For this review, take the finished solid that the model builds, in its own axes (mm). A direction names the side the tool comes from. Give positions to 0.01 mm unless a question says otherwise; leave off trailing zeros. Loops run counter-clockwise (first coordinate to the right, second up) from the corner with the lowest first, then second, coordinate; pieces in that order, holes last. Notation, with made-up numbers: (87, 74) - (106, 74) arc R27 cw to (106, 102) - close; hole circle Ø7 at (1, 60). An arc over 180 degrees is marked (long way). Answer as CSV lines item,"result".
from build123d import *

# Parameters (mm, degrees)
SKETCH1_R           = 12.5
BOSS_EXTRUDE1_DEPTH = 5
SKETCH2_R           = 10
BOSS_EXTRUDE2_DEPTH = 20
CUT_EXTRUDE2_DEPTH  = 3


with BuildPart() as part:
    # Sketch1 → Boss-Extrude1 (new body)
    with BuildSketch(Plane.XY):
        Circle(SKETCH1_R)
    extrude(amount=BOSS_EXTRUDE1_DEPTH)

    # Sketch2 → Boss-Extrude2 (add)
    with BuildSketch(Plane.XY.offset(5)):
        Circle(SKETCH2_R)
    extrude(amount=BOSS_EXTRUDE2_DEPTH)

    # Sketch3 → Cut-Extrude2 (cut)
    with BuildSketch(Plane(origin=(0, 0, 0), x_dir=(-1, 0, 0), z_dir=(0, 0, -1))):
        with BuildLine():
            Line((1.83229916, 12.364977953), (1.83229916, -12.364977953))
            ThreePointArc((1.83229916, -12.364977953), (0, -12.5), (-1.83229916, -12.364977953))
            Line((-1.83229916, -12.364977953), (-1.83229916, 12.364977953))
            ThreePointArc((-1.83229916, 12.364977953), (0, 12.5), (1.83229916, 12.364977953))
        make_face()
    extrude(amount=-CUT_EXTRUDE2_DEPTH, mode=Mode.SUBTRACT)


solid = part.part
1) Consider section A-A on y = 0. Write out the cut boundary in (x, z), and give its area (3 significant figures).
From the geometry:
outline,"(-12.5, 0) - (-1.83, 0) - (-1.83, 3) - (1.83, 3) - (1.83, 0) - (12.5, 0) - (12.5, 5) - (10, 5) - (10, 25) - (-10, 25) - (-10, 5) - (-12.5, 5) - close"
area,"514 mm^2"
2) Consider section C-C on z = 21.5. Write out the cut boundary in (x, y), and give its area (3 significant figures).
From the geometry:
outline,"circle Ø20 at (0, 0)"
area,"314 mm^2"
3) Insertion check: P1, Ø10, axis at y = -6.5, z = 7.5, coming from the +X side; P2, Ø3, axis at y = 6.5, z = 17, coming from the +X side; P3, Ø3.5, axis at y = 2, z = 1, coming from the +X side. Each pin has a flat end and moves straight along its axis. Give the tip position at first contact, or say it passes through.
From the geometry:
P1,"stops at x = 12.31"
P2,"stops at x = 8.66"
P3,"stops at x = 12.5"
4) Wall thickness on line 1 (Z direction, x = 9.75, y = -4.25); line 2 (X direction, y = 11, z = 1); line 3 (X direction, y = -4.25, z = 10.75): over which ranges is each line inside the solid? List them lowest first. Write a range as from..to.
From the geometry:
line 1,"z = 0..5"
line 2,"x = -5.94..-1.83, 1.83..5.94"
line 3,"x = -9.05..9.05"
5) Draft analysis for pull direction X (two halves, no side actions). For faces 4 (the cylindrical face through (-2.71, -12.203, 2.465)), 5 (the flat face through (6, 0, 0)), 6 (the flat face through (-1.832, 0, 1)), state which applies: pulls with the +X half, pulls with the -X half, needs draft (parallel to the pull), parting line crosses it, or undercut.
From the geometry:
face 4,"parting line crosses it"
face 5,"needs draft"
face 6,"undercut"
6) Machinability: for faces 1 (the flat face through (0, 0, 25)), 2 (the flat face through (1.832, 0, 1)), 3 (the flat face through (-0.1, 10.2, 5)), which of the approach directions +Z, -Z, +X, -X, +Y, -Y give a long, thin tool a straight path to every point of the face, cutting with its end or side? Answer none if there is none.
From the geometry:
face 1,"+Z, +X, -X, +Y, -Y"
face 2,"-Z, +Y, -Y"
face 3,"+Z"
7) Consider section D-D on x = 8.5. Write out the cut boundary in (y, z).
From the geometry:
outline,"(-9.17, 0) - (9.17, 0) - (9.17, 5) - (5.27, 5) - (5.27, 25) - (-5.27, 25) - (-5.27, 5) - (-9.17, 5) - close"
8) Consider section B-B on x = 0. Write out the cut boundary in (y, z).
From the geometry:
outline,"(-12.5, 3) - (12.5, 3) - (12.5, 5) - (10, 5) - (10, 25) - (-10, 25) - (-10, 5) - (-12.5, 5) - close"
